```python
from build123d import *

# Parameters (mm, degrees)
CHAMFER1_SIZE       = 2
CUT_EXTRUDE1_DEPTH  = 88
BOSS_EXTRUDE1_DEPTH = 13.5
SCALE_1_SCALE       = 1.875


with BuildPart() as part:
    # Sketch1 → Revolve1 (revolve)
    with BuildSketch(Plane.XY, mode=Mode.PRIVATE) as revolve1_sk:
        Polygon((-66.093473684, 0), (-66.093473684, 17.5), (-31.093473684, 17.5), (-31.093473684, 18.5), (11.906526316, 18.5), (11.906526316, 22.5), (21.906526316, 22.5), (21.906526316, 18.5), (79.906526316, 18.5), (79.906526316, 17.5), (111.906526316, 17.5), (111.906526316, 0), align=None)
    revolve(revolve1_sk.sketch.rotate(Axis((-66.093473684, 0, 0), (1, 0, 0)), 90), axis=Axis((-66.093473684, 0, 0), (1, 0, 0)))

    # Chamfer1
    chamfer1_edges = [part.edges().sort_by_distance(p)[0] for p in [
        (-66.093473684, 0, -17.5),
        (111.906526316, 0, -17.5),
    ]]
    chamfer(chamfer1_edges, length=CHAMFER1_SIZE)

    # Sketch 2_2 → Cut-Extrude1 (cut)
    with BuildSketch(Plane(origin=(0, 0, 0), x_dir=(1, 0, 0), z_dir=(0, 1, 0))):
        with BuildLine():
            Line((-21.093473684, 4.5), (-0.093473684, 4.5))
            ThreePointArc((-0.093473684, 4.5), (4.406526316, 0), (-0.093473684, -4.5))
            Line((-0.093473684, -4.5), (-21.093473684, -4.5))
            ThreePointArc((-21.093473684, -4.5), (-25.593473684, 0), (-21.093473684, 4.5))
        make_face()
        with BuildLine():
            Line((34.906526316, 4.5), (69.906526316, 4.5))
            ThreePointArc((69.906526316, 4.5), (74.406526316, 0), (69.906526316, -4.5))
            Line((69.906526316, -4.5), (34.906526316, -4.5))
            ThreePointArc((34.906526316, -4.5), (30.406526316, 0), (34.906526316, 4.5))
        make_face()
    extrude(amount=-CUT_EXTRUDE1_DEPTH, mode=Mode.SUBTRACT)

    # Sketch 2_2 2 → Boss-Extrude1 (add)
    with BuildSketch(Plane(origin=(0, 0, 0), x_dir=(1, 0, 0), z_dir=(0, 1, 0))):
        with BuildLine():
            Line((-21.093473684, 4.5), (-0.093473684, 4.5))
            ThreePointArc((-0.093473684, 4.5), (4.406526316, 0), (-0.093473684, -4.5))
            Line((-0.093473684, -4.5), (-21.093473684, -4.5))
            ThreePointArc((-21.093473684, -4.5), (-25.593473684, 0), (-21.093473684, 4.5))
        make_face()
        with BuildLine():
            Line((34.906526316, 4.5), (69.906526316, 4.5))
            ThreePointArc((69.906526316, 4.5), (74.406526316, 0), (69.906526316, -4.5))
            Line((69.906526316, -4.5), (34.906526316, -4.5))
            ThreePointArc((34.906526316, -4.5), (30.406526316, 0), (34.906526316, 4.5))
        make_face()
    extrude(amount=-BOSS_EXTRUDE1_DEPTH)


with BuildPart() as part_1:
    # Scale 1: scaled about (22.77118049, 0.261331354, 1.672e-06)
    add(part.part.scale(SCALE_1_SCALE).moved(Location((-19.924782929, -0.228664935, -1.463e-06))))


solid = part_1.part
```
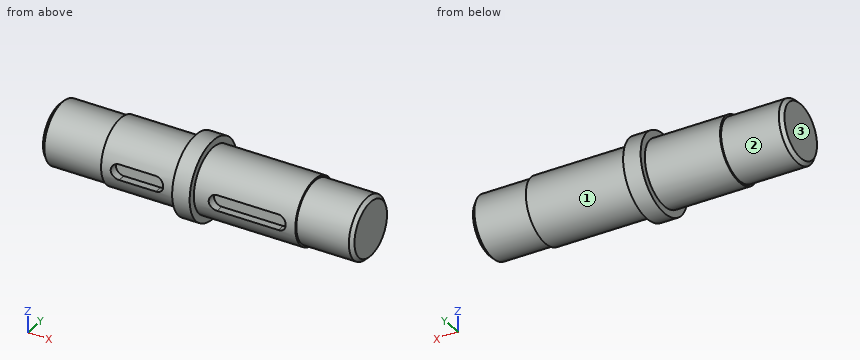
The model under review builds one solid part; all positions refer to its coordinate system, in mm. Face numbers are marked on the shaded views. A direction names the side the tool comes from. Give positions to 0.01 mm unless a question says otherwise; leave off trailing zeros. Order: outer loops, then holes, each group sorted by start corner. A loop starts at its lowest first (then second) coordinate and runs counter-clockwise, first axis right, second up. Notation, with made-up numbers: (54, -28) - (60, -28) arc R23 cw to (60, -4) - close; hole circle Ø7 at (78, 13). An arc over 180 degrees is marked (long way). Use CSV: the item, a comma, the result in double quotes. Start each with the question number.
Q1. We need section C-C, the plane x = -103.5. Write out the cut boundary in (y, z) (1 decimal), and give its area (3 significant figures).
Q2. We need section A-A, the plane x = 51.5. Write out the cut boundary in (y, z) (1 decimal).
Q3. Clearance check with flat-ended pins moving along their axes: pin 1 Ø9 at (x, y) = (91, -30) entering from -Z; pin 2 Ø9 at (x, y) = (-48, -28) entering from +Z; pin 3 Ø6.5 at (x, y) = (69, -29.5) entering from +Z. State where each tip first meets the part, or that it passes through.
Q4. To check wall thickness, follow line 1 along X through (y, z) = (-22, -26.5); line 2 along X through (y, z) = (21.5, 36); line 3 along Y through (x, z) = (-104.5, 0). State the ranges of each line that lie inside material, in increasing order. Write a range as [from, to].
Q5. We need section B-B, the plane x = -7.5. Write out the cut boundary in (y, z) (1 decimal).
Q6. Tool access review of the marked faces 1, 2 and 3: name each direction out of +Z, -Z, +X, -X, +Y, -Y from which nothing blocks a thin tool from reaching the whole face with its end or side.
Outcome:
1,outline,"circle Ø65.6 at (-0.2, 0)"
1,area,"3,380 mm^2"
2,outline,"(-33.9, -8.4) arc R34.7 ccw (long way) to (-33.9, 8.4) - (-25.5, 8.4) - (-25.5, -8.4) - close"
3,pin 1,"stops at z = -23.76"
3,pin 2,"stops at z = 25.72"
3,pin 3,"stops at z = 22.94"
4,line 1,"x = [-78.23, 129.9]"
4,line 2,"x = [2.4, 21.15]"
4,line 3,"y = [-33.04, 32.58]"
5,outline,"circle Ø69.4 at (-0.2, 0)"
6,face 1,"+X"
6,face 2,"-X"
6,face 3,"+Z, -Z, -X, +Y, -Y"
